Check sheet for the modelled part. Datum: model origin and axes. Units: mm. Face numbers are marked on the shaded views. A direction names the side the tool comes from. Coordinates: 2 decimals unless noted, no trailing zeros. Write each loop counter-clockwise with the first axis right and the second up, starting at its lowest first coordinate (ties: lowest second). Pieces come first, ordered by that corner, then holes. Notation, with made-up numbers: M -30.75,10.5 L -22.75,10.5 A15 ccw -22.75,19.5 Z; hole C 3.25,19.5 d3. An arc over 180 degrees is marked long. Answer as CSV lines item,"result".
from build123d import *
from OCP.BRepFilletAPI import BRepFilletAPI_MakeChamfer

# Parameters (mm, degrees)
EXTRUDE_1_DEPTH          = 246.5
CUT_EXTRUDE_1_DEPTH      = 263.865459884
CUT_EXTRUDE_1_DEPTH_BACK = 263.865459884
CHAMFER_1_SIZE           = 6
CHAMFER_1_SIZE2          = 7.103434065
CHAMFER_1_SIZE2_2        = 6.742931709


with BuildPart() as part:
    # 草图1 → 凸台-拉伸1 (new, symmetric)
    with BuildSketch(Plane.XY):
        Polygon((44, 80), (-44, 80), (-44, 76), (-3, 72), (-3, -72), (-44, -76), (-44, -80), (44, -80), (44, -76), (3, -72), (3, 72), (44, 76), align=None)
    extrude(amount=EXTRUDE_1_DEPTH, both=True)

    # 草图3 → 切除-拉伸1 (cut, two sides: drawn at the far end of the back side and taken through both)
    with BuildSketch(Plane(origin=(0, 0, 0), x_dir=(0, 0, -1), z_dir=(1, 0, 0)).offset(-CUT_EXTRUDE_1_DEPTH_BACK)):
        Polygon((-246.5, 66), (-189.5, 72), (-189.5, 80), (-246.5, 80), align=None)
        Polygon((246.5, 80), (246.5, 66), (205.5, 72), (205.5, 80), align=None)
        Polygon((246.5, -66), (205.5, -72), (205.5, -80), (246.5, -80), align=None)
        Polygon((-246.5, -80), (-246.5, -66), (-189.5, -72), (-189.5, -80), align=None)
    extrude(amount=CUT_EXTRUDE_1_DEPTH + CUT_EXTRUDE_1_DEPTH_BACK, mode=Mode.SUBTRACT)

    # 倒角1: one chamfer whose edges measure the first distance from different faces: ONE call of the kernel's chamfer builder (chamfer() names one face for all edges)
    chamfer_1_edges_1 = [part.edges().sort_by_distance(p)[0] for p in [
        (0, 66, -246.5),
        (0, -66, -246.5),
    ]]
    chamfer_1_side_1 = [part.faces().sort_by_distance(p)[0] for p in [
        (0, 0, -246.5),
    ]]
    chamfer_1_edges_2 = [part.edges().sort_by_distance(p)[0] for p in [
        (0, 66, 246.5),
    ]]
    chamfer_1_side_2 = [part.faces().sort_by_distance(p)[0] for p in [
        (0, 69, 218),
    ]]
    chamfer_1_edges_3 = [part.edges().sort_by_distance(p)[0] for p in [
        (0, -66, 246.5),
    ]]
    chamfer_1_side_3 = [part.faces().sort_by_distance(p)[0] for p in [
        (0, -69, 218),
    ]]
    chamfer_1 = BRepFilletAPI_MakeChamfer(part.part.solid().wrapped)
    for e in chamfer_1_edges_1:
        chamfer_1.Add(CHAMFER_1_SIZE, CHAMFER_1_SIZE2, e.wrapped, chamfer_1_side_1[0].wrapped)  # the first distance lies on this face
    for e in chamfer_1_edges_2:
        chamfer_1.Add(CHAMFER_1_SIZE, CHAMFER_1_SIZE2_2, e.wrapped, chamfer_1_side_2[0].wrapped)  # the first distance lies on this face
    for e in chamfer_1_edges_3:
        chamfer_1.Add(CHAMFER_1_SIZE, CHAMFER_1_SIZE2_2, e.wrapped, chamfer_1_side_3[0].wrapped)  # the first distance lies on this face
    add(Compound.cast(chamfer_1.Shape()), mode=Mode.REPLACE)


solid = part.part
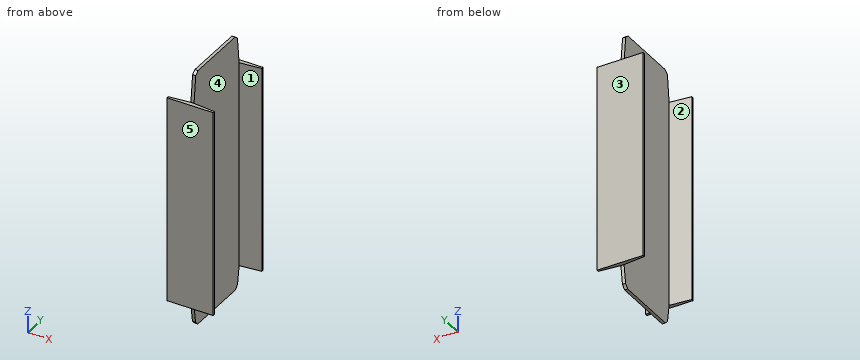
1) Section check B-B, the plane z = -115. Record the boundary of the cut face in (x, y), plus the area to 3 significant figures.
Answer key:
outline,"M -44,-80 L 44,-80 L 44,-76 L 3,-72 L 3,72 L 44,76 L 44,80 L -44,80 L -44,76 L -3,72 L -3,-72 L -44,-76 Z"
area,"1,940 mm2"
2) Depth check by flat-ended pin: P1, Ø4, axis at y = 16, z = 8.5, coming from the +X side; P2, Ø4, axis at x = -3.5, y = -77, coming from the -Z side; P3, Ø4, axis at x = -2.5, y = -75, coming from the +Z side. Enter the tip coordinate at first touch or a pass-through.
Answer key:
P1,"stops at x = 3"
P2,"stops at z = -205.5"
P3,"stops at z = 189.5"
3) Thickness scan on line 1 along X through (y, z) = (-32, 128); line 2 along Y through (x, z) = (4.5, 106.5); line 3 along Y through (x, z) = (-27, -150). Record the ranges inside material, lowest first.
Answer key:
line 1,"x = -3 to 3"
line 2,"y = -80 to -72.15, 72.15 to 80"
line 3,"y = -80 to -74.34, 74.34 to 80"
4) Section check D-D, the plane x = -21.5. Record the boundary of the cut face in (y, z), plus the area to 3 significant figures.
Answer key:
outline,"M -80,-205.5 L -73.8,-205.5 L -73.8,189.5 L -80,189.5 Z; M 73.8,-205.5 L 80,-205.5 L 80,189.5 L 73.8,189.5 Z"
area,"4,890 mm2"
5) Tool access check on the marked faces 1 and 2. Record the directions out of +Z, -Z, +X, -X, +Y, -Y that give a thin tool (end or side, any length) a straight path to the whole face; none if there is none.
Answer key:
face 1,"+Z, -Z, +X"
face 2,"+Z, -Z, -X"
6) Section check C-C, the plane y = -10. Record the boundary of the cut face in (x, z).
Answer key:
outline,"M -3,-246.5 L 3,-246.5 L 3,246.5 L -3,246.5 Z"
7) Mould release check, pull along Y, two halves, no side actions. Record for the marked faces 3, 4 and 5: pulls with the +Y half, pulls with the -Y half, needs draft (parallel to the pull), parting line crosses it, or undercut.
Answer key:
face 3,"pulls with the +Y half"
face 4,"undercut"
face 5,"pulls with the -Y half"
8) Section check A-A, the plane x = 14. Record the boundary of the cut face in (y, z), plus the area to 3 significant figures.
Answer key:
outline,"M -80,-205.5 L -73.07,-205.5 L -73.07,189.5 L -80,189.5 Z; M 73.07,-205.5 L 80,-205.5 L 80,189.5 L 73.07,189.5 Z"
area,"5,470 mm2"
